The listing builds one solid part. Answer for the finished solid, in the listing's coordinates (mm). Give positions to 0.01 mm unless a question says otherwise; leave off trailing zeros. Loops run counter-clockwise (first coordinate to the right, second up) from the corner with the lowest first, then second, coordinate; pieces in that order, holes last. Notation, with made-up numbers: M 69,-33.5 L 76,-33.5 A14 cw 76,-7.5 Z; hole C 80,7.25 d7. An arc over 180 degrees is marked long. One line per item, written item: value. Start each with the question number.
Q1. A cutting plane is placed at B-B, the plane z = -12.5. Determine the outline of the cut face in (x, y), and give its area (3 significant figures).
Q2. Consider L1, parallel to Z at x = 22.5, y = -3.75; L2, parallel to Z at x = 22.5, y = 2.15; L3, parallel to X at y = -0.5, z = 24.5. Determine where each line is inside the solid, lowest interval first.
Q3. Flat-ended cylindrical pins translate along their axes: pin 1 (5 mm diameter, centred on x = 10, z = 12.5, fed in from +Y); pin 2 (2.5 mm diameter, centred on x = 21.5, y = 0, fed in from +Z); pin 3 (6 mm diameter, centred on x = 22.5, z = 16, fed in from +Y); pin 4 (5 mm diameter, centred on x = 11, z = -11.5, fed in from -Y). Find the tip coordinate at first contact, or state that the pin passes through.
Q4. A cutting plane is placed at D-D, the plane y = 3.75. Determine the outline of the cut face in (x, z), and give its area (3 significant figures).
Q5. A cutting plane is placed at C-C, the plane x = -22.5. Determine the outline of the cut face in (y, z), and give its area (3 significant figures).
Q6. A cutting plane is placed at A-A, the plane z = -26. Determine the outline of the cut face in (x, y).
from build123d import *

# Parameters (mm, degrees)
SKETCH_1_W                   = 60
SKETCH_1_H                   = 65
EXTRUDE_1_DEPTH              = 5
HOLE_WIZARD_M5_1_D           = 5.5
HOLE_WIZARD_M5_1_CBORE_D     = 10
HOLE_WIZARD_M5_1_CBORE_DEPTH = 5.4
F_5_0MM_1_D                  = 5
F_5_0MM_1_DEPTH              = 7
HOLE_WIZARD_M5_1_2_D         = 4.2
HOLE_WIZARD_M5_1_2_DEPTH     = 12.4
HOLE_WIZARD_M5_1_2_TIP       = 1.2618073
HOLE_WIZARD_M5_2_D           = 5.5
HOLE_WIZARD_M5_2_CBORE_D     = 10
HOLE_WIZARD_M5_2_CBORE_DEPTH = 5.4


with BuildPart() as part:
    # 草图1 → 凸台-拉伸1 (new, symmetric)
    with BuildSketch(Plane(origin=(0, 0, 0), x_dir=(1, 0, 0), z_dir=(0, 1, 0))):
        Rectangle(SKETCH_1_W, SKETCH_1_H)
    extrude(amount=EXTRUDE_1_DEPTH, both=True)

    # Hole Wizard M5 _1 (through all)
    with Locations(Plane(origin=(0, 5, 0), x_dir=(1, 0, 0), z_dir=(0, 1, 0))):
        with Locations((-22.5, 26), (-22.5, -16), (22.5, -16), (22.5, 26)):
            CounterBoreHole(HOLE_WIZARD_M5_1_D / 2, HOLE_WIZARD_M5_1_CBORE_D / 2, HOLE_WIZARD_M5_1_CBORE_DEPTH)

    # Ø5.0mm 暗销孔1
    with Locations(Plane.XY.offset(32.5)):
        with Locations((-22.5, 0), (22.5, 0)):
            Hole(F_5_0MM_1_D / 2, depth=F_5_0MM_1_DEPTH)

    # Hole Wizard M5 _1 2
    with Locations(Plane.XY.offset(32.5)):
        with Locations((-13, 0), (13, 0)):
            Hole(HOLE_WIZARD_M5_1_2_D / 2, depth=HOLE_WIZARD_M5_1_2_DEPTH)
            with Locations((0, 0, -(HOLE_WIZARD_M5_1_2_DEPTH + HOLE_WIZARD_M5_1_2_TIP / 2))):  # 118° drill point
                Cone(0, HOLE_WIZARD_M5_1_2_D / 2, HOLE_WIZARD_M5_1_2_TIP, mode=Mode.SUBTRACT)

    # M5 六角凹头螺钉的柱形沉头孔2 (through all)
    with Locations(Plane(origin=(0, -5, 0), x_dir=(-1, 0, 0), z_dir=(0, -1, 0))):
        with Locations((-10, -12.5), (-10, 12.5)):
            CounterBoreHole(HOLE_WIZARD_M5_2_D / 2, HOLE_WIZARD_M5_2_CBORE_D / 2, HOLE_WIZARD_M5_2_CBORE_DEPTH)


solid = part.part
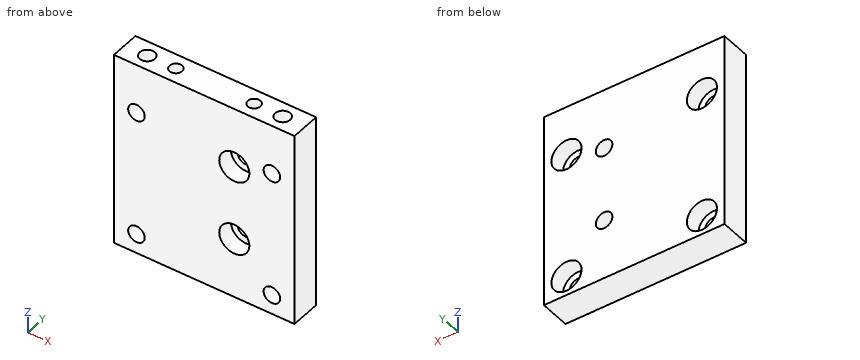
Answer block:
1. outline: M -30,-5 L 5,-5 L 5,0.4 L 7.25,0.4 L 7.25,5 L -30,5 Z; M 12.75,0.4 L 15,0.4 L 15,-5 L 30,-5 L 30,5 L 12.75,5 Z
1. area: 521 mm^2
2. L1: -32.5 to -28.75, -23.25 to 13.25, 18.75 to 32.5
2. L2: -32.5 to -31, -21 to 11, 21 to 25.5
2. L3: -30 to -15.04, -10.96 to 10.96, 15.04 to 30
3. pin 1: through
3. pin 2: z = 25.5
3. pin 3: y = -0.4
3. pin 4: y = 0.4
4. outline: M -30,-32.5 L 30,-32.5 L 30,32.5 L -30,32.5 Z; hole C -22.5,-26 d10; hole C -22.5,16 d10; hole C 10,-12.5 d5.5; hole C 10,12.5 d5.5; hole C 22.5,-26 d10; hole C 22.5,16 d10
4. area: 3,540 mm^2
5. outline: M -5,-32.5 L 5,-32.5 L 5,-31 L -0.4,-31 L -0.4,-28.75 L -5,-28.75 Z; M -5,-23.25 L -0.4,-23.25 L -0.4,-21 L 5,-21 L 5,11 L -0.4,11 L -0.4,13.25 L -5,13.25 Z; M -5,18.75 L -0.4,18.75 L -0.4,21 L 5,21 L 5,32.5 L 2.5,32.5 L 2.5,25.5 L -2.5,25.5 L -2.5,32.5 L -5,32.5 Z
5. area: 456 mm^2
6. outline: M -30,-5 L -25.25,-5 L -25.25,-0.4 L -27.5,-0.4 L -27.5,5 L -30,5 Z; M -19.75,-5 L 19.75,-5 L 19.75,-0.4 L 17.5,-0.4 L 17.5,5 L -17.5,5 L -17.5,-0.4 L -19.75,-0.4 Z; M 25.25,-5 L 30,-5 L 30,5 L 27.5,5 L 27.5,-0.4 L 25.25,-0.4 Z
